```python
from build123d import *

# Parameters (mm, degrees)
SKETCH_1_R      = 1.5
EXTRUDE_1_DEPTH = 3


with BuildPart() as part:
    # 草图1 → 凸台-拉伸1 (new body)
    with BuildSketch(Plane.XY):
        with BuildLine():
            ThreePointArc((-3.035621948, 26.828809131), (-3.826001677, 25.273746937), (-5.347923635, 24.421296296))
            ThreePointArc((-5.347923635, 24.421296296), (-17.67766953, 17.67766953), (-24.421296296, 5.347923635))
            ThreePointArc((-24.421296296, 5.347923635), (-25.403311193, 3.708624428), (-27.175925926, 2.994837236))
            ThreePointArc((-27.175925926, 2.994837236), (-30, 0), (-27.175925926, -2.994837236))
            ThreePointArc((-27.175925926, -2.994837236), (-25.403311193, -3.708624428), (-24.421296296, -5.347923635))
            ThreePointArc((-24.421296296, -5.347923635), (-17.67766953, -17.67766953), (-5.347923635, -24.421296296))
            ThreePointArc((-5.347923635, -24.421296296), (-3.708624428, -25.403311193), (-2.994837236, -27.175925926))
            ThreePointArc((-2.994837236, -27.175925926), (0, -30), (2.994837236, -27.175925926))
            ThreePointArc((2.994837236, -27.175925926), (3.708624428, -25.403311193), (5.347923635, -24.421296296))
            ThreePointArc((5.347923635, -24.421296296), (17.67766953, -17.67766953), (24.421296296, -5.347923635))
            ThreePointArc((24.421296296, -5.347923635), (25.403311193, -3.708624428), (27.175925926, -2.994837236))
            ThreePointArc((27.175925926, -2.994837236), (30, 0), (27.175925926, 2.994837236))
            ThreePointArc((27.175925926, 2.994837236), (25.403311193, 3.708624428), (24.421296296, 5.347923635))
            ThreePointArc((24.421296296, 5.347923635), (17.67766953, 17.67766953), (5.347923635, 24.421296296))
            ThreePointArc((5.347923635, 24.421296296), (3.826001677, 25.273746937), (3.035621948, 26.828809131))
            ThreePointArc((3.035621948, 26.828809131), (3.015495219, 26.831078782), (2.995366793, 26.833333333))
            ThreePointArc((2.995366793, 26.833333333), (2.999996416, 27.004637195), (2.994837236, 27.175925926))
            ThreePointArc((2.994837236, 27.175925926), (0, 30), (-2.994837236, 27.175925926))
            ThreePointArc((-2.994837236, 27.175925926), (-2.999996416, 27.004637195), (-2.995366793, 26.833333333))
            ThreePointArc((-2.995366793, 26.833333333), (-3.015495219, 26.831078782), (-3.035621948, 26.828809131))
        make_face()
        with Locations((-27, 0)):
            Circle(SKETCH_1_R, mode=Mode.SUBTRACT)
        with Locations((0, -27)):
            Circle(SKETCH_1_R, mode=Mode.SUBTRACT)
        with Locations((27, 0)):
            Circle(SKETCH_1_R, mode=Mode.SUBTRACT)
        with Locations((0, 27)):
            Circle(SKETCH_1_R, mode=Mode.SUBTRACT)
    extrude(amount=EXTRUDE_1_DEPTH)


solid = part.part
```
Source: CAD feature listing. Evaluate the final solid. Frame: model axes, mm. Give positions to 0.01 mm unless a question says otherwise; leave off trailing zeros. Loops run counter-clockwise (first coordinate to the right, second up) from the corner with the lowest first, then second, coordinate; pieces in that order, holes last. Notation, with made-up numbers: (38.5, -18.5) -> (66.5, -18.5) arc R23 ccw to (66.5, 6.5) -> close; hole circle Ø5 at (73, 24). An arc over 180 degrees is marked (long way). Use a Markdown table: item, result. Add a question column.
(1) Pull-direction query (Y, two-part tool) for faces 1 (the face through (-28.5, 0.07, 1.48)), 2 (the face through (0, 0, 3)), 3 (the face through (17.536, -17.818, 1.479)); classes: +Y half, -Y half, draft (parallel to the pull), parting line (faces both ways), or undercut.
(2) Ray query, line 1 (Y direction, x = 0, z = 1.3); line 2 (Y direction, x = 27, z = 1.7); line 3 (Y direction, x = 26.5, z = 2.2). Return the intervals inside material, ascending.
(3) Section query B-B (z = 1.5). Output: boundary loops of the cut face in (x, y), then the cut area to 3 significant figures.
(4) Section query D-D (y = -7). Output: boundary loops of the cut face in (x, z), then the cut area to 3 significant figures.
(5) Section query A-A (x = 0). Output: boundary loops of the cut face in (y, z), then the cut area to 3 significant figures.
Checked values:
| question | item | result |
|---|---|---|
| 1 | face 1 | undercut |
| 1 | face 2 | draft |
| 1 | face 3 | -Y half |
| 2 | line 1 | -30 to -28.5, -25.5 to 25.5, 28.5 to 30 |
| 2 | line 2 | -3.01 to -1.5, 1.5 to 3.01 |
| 2 | line 3 | -3.11 to -1.41, 1.41 to 3.11 |
| 3 | outline | (-27.18, -2.99) arc R3 cw to (-24.42, -5.35) arc R25 ccw to (-5.35, -24.42) arc R3 cw to (-2.99, -27.18) arc R3 ccw to (2.99, -27.18) arc R3 cw to (5.35, -24.42) arc R25 ccw to (24.42, -5.35) arc R3 cw to (27.18, -2.99) arc R3 ccw to (27.18, 2.99) arc R3 cw to (24.42, 5.35) arc R25 ccw to (5.35, 24.42) arc R3 cw to (3.04, 26.83) arc R27 ccw to (3, 26.83) arc R3 ccw (long way) to (-3, 26.83) arc R27 ccw to (-3.04, 26.83) arc R3 cw to (-5.35, 24.42) arc R25 ccw to (-24.42, 5.35) arc R3 cw to (-27.18, 2.99) arc R3 ccw to start; hole circle Ø3 at (-27, 0); hole circle Ø3 at (0, -27); hole circle Ø3 at (0, 27); hole circle Ø3 at (27, 0) |
| 3 | area | 2,050 mm^2 |
| 4 | outline | (-24, 0) -> (24, 0) -> (24, 3) -> (-24, 3) -> close |
| 4 | area | 144 mm^2 |
| 5 | outline | (-30, 0) -> (-28.5, 0) -> (-28.5, 3) -> (-30, 3) -> close; (-25.5, 0) -> (25.5, 0) -> (25.5, 3) -> (-25.5, 3) -> close; (28.5, 0) -> (30, 0) -> (30, 3) -> (28.5, 3) -> close |
| 5 | area | 162 mm^2 |
